```python
from build123d import *

# Parameters (mm, degrees)
SKETCH_1_W                  = 50
SKETCH_1_H                  = 20
EXTRUDE_1_DEPTH             = 13.4
SKETCH_2_R                  = 6.2
EXTRUDE_2_DEPTH             = 16
SKETCH_3_R                  = 6.2
EXTRUDE_3_DEPTH             = 16
HOLE_WIZARD_6_0_6_1_D       = 6
HOLE_WIZARD_6_0_6_1_DEPTH   = 30
HOLE_WIZARD_6_0_6_1_TIP     = 1.802581857
HOLE_WIZARD_6_0_6_2_D       = 6
HOLE_WIZARD_6_0_6_2_DEPTH   = 30
HOLE_WIZARD_6_0_6_2_TIP     = 1.802581857
HOLE_WIZARD_4_3_4_3_1_D     = 4.3
HOLE_WIZARD_4_3_4_3_1_DEPTH = 30
HOLE_WIZARD_4_3_4_3_1_TIP   = 1.291850331
FILLET_1_R                  = 2
CUT_EXTRUDE_1_REACH         = 52.364
PATTERN_LINEAR_1_COUNT      = 4
PATTERN_LINEAR_1_PITCH      = 5
CUT_EXTRUDE_2_REACH         = 52.364
PATTERN_LINEAR_2_COUNT      = 3
PATTERN_LINEAR_2_PITCH      = 5


with BuildPart() as part:
    # 草图1 → 凸台-拉伸1 (new body)
    with BuildSketch(Plane.XY):
        Rectangle(SKETCH_1_W, SKETCH_1_H)
    extrude(amount=EXTRUDE_1_DEPTH)

    # 草图2 → 凸台-拉伸2 (add)
    with BuildSketch(Plane.XZ.offset(10)):
        with Locations(Location((-13.5, 6.7, 0), (0, 0, 90))):
            Circle(SKETCH_2_R)
    extrude(amount=EXTRUDE_2_DEPTH)

    # 草图3 → 凸台-拉伸3 (add)
    with BuildSketch(Plane.ZY.offset(25)):
        with Locations(Location((6.7, 0, 0), (0, 0, 180))):
            Circle(SKETCH_3_R)
    extrude(amount=EXTRUDE_3_DEPTH)

    # Ø6.0 (6) 直径孔1
    with Locations(Plane.ZY.offset(41)):
        with Locations((6.7, 0)):
            Hole(HOLE_WIZARD_6_0_6_1_D / 2, depth=HOLE_WIZARD_6_0_6_1_DEPTH)
            with Locations((0, 0, -(HOLE_WIZARD_6_0_6_1_DEPTH + HOLE_WIZARD_6_0_6_1_TIP / 2))):  # 118° drill point
                Cone(0, HOLE_WIZARD_6_0_6_1_D / 2, HOLE_WIZARD_6_0_6_1_TIP, mode=Mode.SUBTRACT)

    # Ø6.0 (6) 直径孔2
    with Locations(Plane.XZ.offset(26)):
        with Locations((-13.5, 6.7)):
            Hole(HOLE_WIZARD_6_0_6_2_D / 2, depth=HOLE_WIZARD_6_0_6_2_DEPTH)
            with Locations((0, 0, -(HOLE_WIZARD_6_0_6_2_DEPTH + HOLE_WIZARD_6_0_6_2_TIP / 2))):  # 118° drill point
                Cone(0, HOLE_WIZARD_6_0_6_2_D / 2, HOLE_WIZARD_6_0_6_2_TIP, mode=Mode.SUBTRACT)

    # Ø4.3 (4.3) 直径孔1
    with Locations(Plane.XY.offset(13.4)):
        with Locations((-20, 6), (-20, -6)):
            Hole(HOLE_WIZARD_4_3_4_3_1_D / 2, depth=HOLE_WIZARD_4_3_4_3_1_DEPTH)
            with Locations((0, 0, -(HOLE_WIZARD_4_3_4_3_1_DEPTH + HOLE_WIZARD_4_3_4_3_1_TIP / 2))):  # 118° drill point
                Cone(0, HOLE_WIZARD_4_3_4_3_1_D / 2, HOLE_WIZARD_4_3_4_3_1_TIP, mode=Mode.SUBTRACT)

    # 圆角1
    fillet_1_edges = [part.edges().sort_by_distance(p)[0] for p in [
        (25, -10, 6.7),
        (-25, -10, 6.7),
        (-25, 10, 6.7),
        (25, 10, 6.7),
    ]]
    fillet(fillet_1_edges, radius=FILLET_1_R)

    # 草图11 → 切除-拉伸1 (cut, up to next)
    with BuildSketch(Plane.XY.offset(13.4), mode=Mode.PRIVATE) as cut_extrude_1_sk1:
        with BuildLine():
            Line((0.3, 8.75), (0.3, 6.25))
            ThreePointArc((0.3, 6.25), (0, 5.95), (-0.3, 6.25))
            Line((-0.3, 6.25), (-0.3, 8.75))
            ThreePointArc((-0.3, 8.75), (0, 9.05), (0.3, 8.75))
        make_face()
    cut_extrude_1_tool1 = extrude(cut_extrude_1_sk1.sketch, amount=-CUT_EXTRUDE_1_REACH, mode=Mode.PRIVATE) & part.part
    cut_extrude_1 = cut_extrude_1_tool1.solids().sort_by_distance((0, 7.5, 13.4))[0]
    add(cut_extrude_1, mode=Mode.SUBTRACT)

    # 阵列(线性)1: 切除-拉伸1 ×4
    with Locations(*[(0, -i * PATTERN_LINEAR_1_PITCH, 0) for i in range(1, PATTERN_LINEAR_1_COUNT)]):
        add(cut_extrude_1, mode=Mode.SUBTRACT)

    # 草图12 → 切除-拉伸2 (cut, up to next)
    with BuildSketch(Plane.XY.offset(13.4), mode=Mode.PRIVATE) as cut_extrude_2_sk1:
        with BuildLine():
            Line((1.8, 6.25), (1.8, 3.75))
            ThreePointArc((1.8, 3.75), (1.5, 3.45), (1.2, 3.75))
            Line((1.2, 3.75), (1.2, 6.25))
            ThreePointArc((1.2, 6.25), (1.5, 6.55), (1.8, 6.25))
        make_face()
    cut_extrude_2_tool1 = extrude(cut_extrude_2_sk1.sketch, amount=-CUT_EXTRUDE_2_REACH, mode=Mode.PRIVATE) & part.part
    cut_extrude_2 = cut_extrude_2_tool1.solids().sort_by_distance((1.5, 5, 13.4))[0]
    add(cut_extrude_2, mode=Mode.SUBTRACT)

    # 阵列(线性)2: 切除-拉伸2 ×3
    with Locations(*[(0, -i * PATTERN_LINEAR_2_PITCH, 0) for i in range(1, PATTERN_LINEAR_2_COUNT)]):
        add(cut_extrude_2, mode=Mode.SUBTRACT)


solid = part.part
```
Can you work these out from the model? Positions are in its coordinate system, mm. A direction names the side the tool comes from. Coordinates: 2 decimals unless noted, no trailing zeros. Order: outer loops, then holes, each group sorted by start corner. A loop starts at its lowest first (then second) coordinate and runs counter-clockwise, first axis right, second up.
1. I'm going to push flat-ended pins straight in: pin 1 (1.5 mm diameter, centred on x = -11.5, y = -18, fed in from -Z); pin 2 (3 mm diameter, centred on y = 0, z = 8, fed in from -X); pin 3 (1.5 mm diameter, centred on x = -30, z = 8.5, fed in from -Y). Where does each tip first touch, or does it pass through?
2. I need wall thicknesses on line 1 (Y direction, x = -20, z = 6.5); line 2 (Z direction, x = -23.5, y = -2.5); line 3 (X direction, y = -2.5, z = 11.75). Which ranges of each line are inside material? Lowest first, please.
3. Thinking about a two-plate mould opening in Z: for faces 1 (the face through (-11.1, 2.9, 4.9)), 2 (the face through (-12, 0, 9.7)), 3 (the face through (0.3, -2, 7)), 4 (the face through (-32.9, -1.9, 0.8)), which applies, +Z half, -Z half, draft (parallel to the pull), parting line (faces both ways), or undercut?
4. If we section it at B-B (x = -35.5): Please give me the cut outline in (y, z), then the cut area to 3 significant figures.
5. For faces 5 (the face through (-25, -4, 1)), 6 (the face through (-0.3, -3, 7)), 7 (the face through (-18.73, -17.89, 10.03)), which set-ups out of +Z, -Z, +X, -X, +Y, -Y let a thin tool reach every point of the face, with its end or its side?
6. If we section it at A-A (y = -21): Please give me the cut outline in (x, z), then the cut area to 3 significant figures.
7. If we section it at C-C (z = 2.5): Give the number of separate pieces and of enclosed holes in the cut face, then the cut area to 3 significant figures.
Entries:
1. pin 1: stops at z = 0.63
1. pin 2: stops at x = -10.88
1. pin 3: stops at y = -6.11
2. line 1: y = -10 to -8.15, -3.85 to -2.99, 2.99 to 3.85, 8.15 to 10
2. line 2: z = 0 to 5.04, 8.36 to 13.4
2. line 3: x = -41 to -0.3, 0.3 to 25
3. face 1: undercut
3. face 2: undercut
3. face 3: draft
3. face 4: parting line
4. outline: circle Ø12.4 at (0, 6.7); hole circle Ø6 at (0, 6.7)
4. area: 92.5 mm2
5. face 5: -X
5. face 6: +Z, -Z
5. face 7: -Y
6. outline: circle Ø12.4 at (-13.5, 6.7); hole circle Ø6 at (-13.5, 6.7)
6. area: 92.5 mm2
7. separate pieces: 1
7. enclosed holes: 9
7. area: 1,250 mm2
